Check sheet for the modelled part. Datum: model origin and axes. Units: mm. A direction names the side the tool comes from. Coordinates: 2 decimals unless noted, no trailing zeros. Loops run counter-clockwise (first coordinate to the right, second up) from the corner with the lowest first, then second, coordinate; pieces in that order, holes last. Notation, with made-up numbers: (61, 27) - (70, 27) arc R23 ccw to (70, 54) - close; hole circle Ø3 at (45.5, 2.25). An arc over 180 degrees is marked (long way). Use a Markdown table: item, result. Add a question column.
1) Sectioned sample at B-B, the plane x = 10. Enter the section's corners in (y, z), then the cut area to 3 significant figures.
2) Draft check along Y on faces 1 (the flat face through (49, 0, 0)), 2 (the flat face through (71, 50, 0)), 3 (the flat face through (49, 17, 8)), 4 (the flat face through (50, 27, -25)). Enter one of: pulls with the +Y half, pulls with the -Y half, needs draft (parallel to the pull), parting line crosses it, or undercut.
3) Go/stop test with flat-tipped pins: P1, Ø4, axis at x = 20.5, y = 41, coming from the +Z side; P2, Ø2, axis at y = 32, z = -15, coming from the -X side (3 decimals); P3, Ø5, axis at x = 43.5, z = 13.5, coming from the +Y side. Record where each tip stops, or that it passes through.
4) Tool access check on faces 5 (the flat face through (49, 17, -8)), 6 (the flat face through (50, 32, -21)), 7 (the cylindrical face through (47.4, 59.83, 0.35)). Record the directions out of +Z, -Z, +X, -X, +Y, -Y that give a thin tool (end or side, any length) a straight path to the whole face; none if there is none.
5) Thickness scan on line 1 (Y direction, x = 26.5, z = -17.5); line 2 (Z direction, x = 75, y = 21); line 3 (X direction, y = 10, z = -2). Record the ranges inside material, lowest first.
6) Sectioned sample at C-C, the plane y = 40. Enter the section's corners in (x, z).
7) Sectioned sample at D-D, the plane z = 4.5. Enter the section's corners in (x, y).
8) Sectioned sample at A-A, the plane z = -14.5. Enter the section's corners in (x, y), then the cut area to 3 significant figures.
from build123d import *

# Parameters (mm, degrees)
BASE_PLATE_DEPTH        = 25
SUPPORT_UPRIGHT_DEPTH   = 8
SHAFT_CYLINDER_SKETCH_R = 20
SHAFT_CYLINDER_40_DEPTH = 25
SHAFT_START             = -8
SHAFT_END_NOTCH_DEPTH   = 8


with BuildPart() as part:
    # Base Plate Sketch → Base Plate (new, symmetric)
    with BuildSketch(Plane.XY):
        Polygon((0, 0), (100, 0), (95, 10), (5, 10), align=None)
    extrude(amount=BASE_PLATE_DEPTH, both=True)

    # Support Upright Sketch → Support Upright (add, symmetric)
    with BuildSketch(Plane.XY):
        Polygon((5, 10), (95, 10), (75, 50), (25, 50), align=None)
    extrude(amount=SUPPORT_UPRIGHT_DEPTH, both=True)

    # Shaft Cylinder Sketch → Shaft Cylinder Ø40 (add, symmetric)
    with BuildSketch(Plane.XY):
        with Locations((50, 40)):
            Circle(SHAFT_CYLINDER_SKETCH_R)
    extrude(amount=SHAFT_CYLINDER_40_DEPTH, both=True)

    # Shaft End Notch Sketch → Shaft End Notch (cut)
    with BuildSketch(Plane(origin=(0, 0, -25), x_dir=(-1, 0, 0), z_dir=(0, 0, -1)).offset(SHAFT_START)):
        with BuildLine():
            Line((-31.66969722, 48), (-68.33030278, 48))
            ThreePointArc((-68.33030278, 48), (-70, 40), (-68.33030278, 32))
            Line((-68.33030278, 32), (-31.66969722, 32))
            ThreePointArc((-31.66969722, 32), (-30, 40), (-31.66969722, 48))
        make_face()
    extrude(amount=SHAFT_END_NOTCH_DEPTH, mode=Mode.SUBTRACT)


solid = part.part
Solved:
| question | item | result |
|---|---|---|
| 1 | outline | (0, -25) - (10, -25) - (10, -8) - (20, -8) - (20, 8) - (10, 8) - (10, 25) - (0, 25) - close |
| 1 | area | 660 mm2 |
| 2 | face 1 | pulls with the -Y half |
| 2 | face 2 | pulls with the +Y half |
| 2 | face 3 | undercut |
| 2 | face 4 | needs draft |
| 3 | P1 | stops at z = 8 |
| 3 | P2 | stops at x = 31.265 |
| 3 | P3 | stops at y = 59.6 |
| 4 | face 5 | -Z |
| 4 | face 6 | -Z, +X, -X |
| 4 | face 7 | none |
| 5 | line 1 | y = 0 to 10 |
| 5 | line 2 | z = -8 to 8 |
| 5 | line 3 | x = 5 to 95 |
| 6 | outline | (20, -8) - (30, -8) - (30, -17) - (70, -17) - (70, -8) - (80, -8) - (80, 8) - (70, 8) - (70, 25) - (30, 25) - (30, 8) - (20, 8) - close |
| 7 | outline | (0, 0) - (100, 0) - (75, 50) - (67.32, 50) arc R20 ccw to (32.68, 50) - (25, 50) - close |
| 8 | outline | (0, 0) - (100, 0) - (95, 10) - (5, 10) - close; circle Ø40 at (50, 40) |
| 8 | area | 2,210 mm2 |
